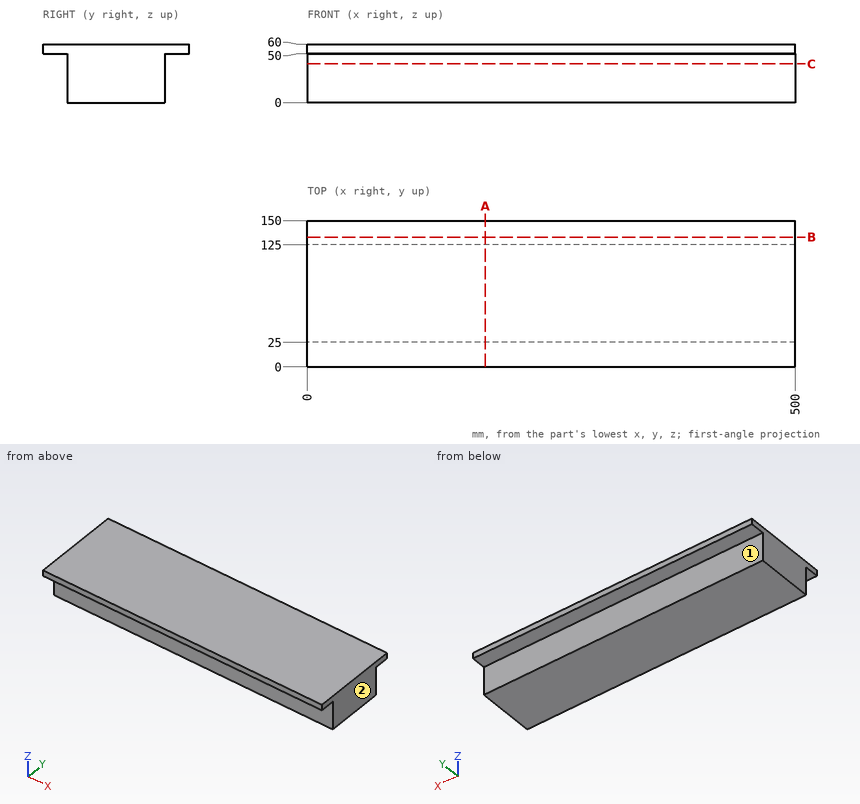
Job drawing, mm, ordinate dimensions from the low corner. One solid piece. A direction names the side the tool comes from. Coordinates: 2 decimals unless noted, no trailing zeros. Order: outer loops, then holes, each group sorted by start corner. A loop starts at its lowest first (then second) coordinate and runs counter-clockwise, first axis right, second up. Notation, with made-up numbers: (40.5, 81.5) -> (58.5, 81.5) arc R16 ccw to (58.5, 101.5) -> close; hole circle Ø2 at (70.25, 18.5). An arc over 180 degrees is marked (long way). Return JSON: item names as keys, results as strings. Group by question number.
Item 1: Wall check: line 1 along Y through (x, z) = (167, 11); line 2 along Z through (x, y) = (38, 141). Give the ranges that are in metal, low to high. Write a range as [from, to].
Item 2: Saw through at A-A on x = 182.5. Write the cut outline in (y, z).
Item 3: Saw through at C-C on z = 39.5. Write the cut outline in (x, y), then the cut area to 3 significant figures.
Item 4: Saw through at B-B on y = 133. Write the cut outline in (x, z), then the cut area to 3 significant figures.
Item 5: Flat gauge pins, fed straight in: P1, Ø20, axis at x = 333.5, y = 142.5, coming from the -Z side; P2, Ø25, axis at x = 130.5, z = 26, coming from the -Y side; P3, Ø1, axis at x = 143.5, z = 17.5, coming from the +Y side. Where does each tip first touch, or does it go through?
Item 6: Tool access for the marked faces 1 and 2: list every direction of +Z, -Z, +X, -X, +Y, -Y with a clear straight run to the whole face (end or side of a thin tool).
Values found:
{
 "1": {"line 1": "y = [25, 125]", "line 2": "z = [50, 60]"},
 "2": {"outline": "(0, 50) -> (25, 50) -> (25, 0) -> (125, 0) -> (125, 50) -> (150, 50) -> (150, 60) -> (0, 60) -> close"},
 "3": {"outline": "(0, 25) -> (500, 25) -> (500, 125) -> (0, 125) -> close", "area": "50,000 mm2"},
 "4": {"outline": "(0, 50) -> (500, 50) -> (500, 60) -> (0, 60) -> close", "area": "5,000 mm2"},
 "5": {"P1": "stops at z = 50", "P2": "stops at y = 25", "P3": "stops at y = 125"},
 "6": {"face 1": "-Z, +X, -X, +Y", "face 2": "+Z, -Z, +X, +Y, -Y"}
}
